from build123d import *

# Parameters (mm, degrees)
BOSS_EXTRUDE1_DEPTH = 6


with BuildPart() as part:
    # Sketch1 → Boss-Extrude1 (new body)
    with BuildSketch(Plane.XY):
        with BuildLine():
            Line((23.424737155, -30.334071959), (17.293543757, -15.098809177))
            ThreePointArc((17.293543757, -15.098809177), (16.817822135, -14.397549548), (16.094423456, -13.956221462))
            Line((16.094423456, -13.956221462), (15.963008089, -14.561962892))
            ThreePointArc((15.963008089, -14.561962892), (16.131735441, -17.04624853), (14.064088238, -15.658812373))
            Line((14.064088238, -15.658812373), (13.483620184, -15.421447711))
            ThreePointArc((13.483620184, -15.421447711), (13.445284936, -16.014246024), (13.582760132, -16.592156052))
            Line((13.582760132, -16.592156052), (19.41043004, -31.073200227))
            Line((19.41043004, -31.073200227), (19.719217872, -30.321121581))
            ThreePointArc((19.719217872, -30.321121581), (21.576335078, -29.08075761), (23.424737155, -30.334071959))
        make_face()
        with BuildLine():
            ThreePointArc((23.419472814, -31.840369211), (23.569333129, -31.087735131), (23.424737155, -30.334071959))
            ThreePointArc((23.424737155, -30.334071959), (21.576335078, -29.08075761), (19.719217872, -30.321121581))
            Line((19.719217872, -30.321121581), (19.41043004, -31.073200227))
            Line((19.41043004, -31.073200227), (19.71395353, -31.827418834))
            ThreePointArc((19.71395353, -31.827418834), (21.562355608, -33.080733182), (23.419472814, -31.840369211))
        make_face()
        with BuildLine():
            Line((18.045273154, -44.929682928), (23.419472814, -31.840369211))
            ThreePointArc((23.419472814, -31.840369211), (21.562355608, -33.080733182), (19.71395353, -31.827418834))
            Line((19.71395353, -31.827418834), (19.41043004, -31.073200227))
            Line((19.41043004, -31.073200227), (14.345018212, -43.410435298))
            Line((14.345018212, -43.410435298), (8.266248414, -50.481735298))
            ThreePointArc((8.266248414, -50.481735298), (14.114121661, -49.393703769), (18.045273154, -44.929682928))
        make_face()
    extrude(amount=BOSS_EXTRUDE1_DEPTH)


solid = part.part
Check sheet for the modelled part. Datum: model origin and axes. Units: mm. A direction names the side the tool comes from. Round coordinates to 2 decimals unless told otherwise and drop trailing zeros. Loops run counter-clockwise (first coordinate to the right, second up) from the corner with the lowest first, then second, coordinate; pieces in that order, holes last. Notation, with made-up numbers: M 65,-40 L 103,-40 A21 ccw 103,-1 Z; hole C 21.25,76 d5. An arc over 180 degrees is marked long. One line per question, with ' | ' between items. Start each with the question number.
Item 1: Gauge pin test, flat ends, axial feed: pin 1 Ø1.7 at (x, y) = (15.44, -15.85) entering from -Z; pin 2 Ø3 at (x, z) = (11.5, 4) entering from +Y; pin 3 Ø2 at (y, z) = (-44.5, 2.5) entering from -X; pin 4 Ø3 at (y, z) = (-46.5, 1.5) entering from +X. Record the tip position at first contact, or that the pin passes through.
Item 2: Section check D-D (y = -47). Record the boundary of the cut face in (x, z), and give its area (3 significant figures).
Item 3: Section check A-A (x = 19). Record the boundary of the cut face in (y, z).
Item 4: Section check C-C (x = 15). Record the boundary of the cut face in (y, z).
Item 5: Section check B-B (z = 2.4). Record the boundary of the cut face in (x, y).
Item 6: Set-up check for faces 5 (the face through (16.456, -23.731, 2.958)), 6 (the face through (16.83, -14.41, 2.96)): record each of +Z, -Z, +X, -X, +Y, -Y from which the full face is reachable in a straight line by a thin tool's end or side.
Item 7: Scan lines: probe 1 along Y at (x, z) = (16.25, 1.7); probe 2 along Y at (x, z) = (15.25, 3.4); probe 3 along Y at (x, z) = (17, 4.4). Record each from-to range of solid material in increasing order.
Item 8: Release check for a two-part mould opening along Y. For faces 1 (the face through (20.695, -38.477, 2.958)), 2 (the face through (20.4, -22.82, 2.96)), 3 (the face through (16.169, -17.024, 2.958)), 4 (the face through (23.57, -31.1, 2.96)) record: released by +Y, released by -Y, zero draft, split by the parting line, or undercut.
Worked out:
1) pin 1: through | pin 2: y = -44.98 | pin 3: x = 12.55 | pin 4: x = 18.02
2) outline: M 11.26,0 L 16.86,0 L 16.86,6 L 11.26,6 Z | area: 33.6 mm^2
3) outline: M -42.6,0 L -32.07,0 L -32.07,6 L -42.6,6 Z; M -30.05,0 L -19.34,0 L -19.34,6 L -30.05,6 Z
4) outline: M -48.82,0 L -41.82,0 L -41.82,6 L -48.82,6 Z; M -20.11,0 L -17.16,0 L -17.16,6 L -20.11,6 Z
5) outline: M 8.27,-50.48 A9.11 ccw 18.05,-44.93 L 23.42,-31.84 A2 ccw 23.42,-30.33 L 17.29,-15.1 A2 ccw 16.09,-13.96 L 15.96,-14.56 A1.39 cw long 14.06,-15.66 L 13.48,-15.42 A2 ccw 13.58,-16.59 L 19.41,-31.07 L 14.35,-43.41 Z
6) face 5: +Z, -Z, -X | face 6: +Z, -Z, +X, +Y
7) probe 1: -47.72 to -38.77, -23.22 to -16.97, -14.72 to -14.02 | probe 2: -48.63 to -41.21, -20.74 to -17.22 | probe 3: -46.81 to -36.94, -25.08 to -14.6
8) face 1: released by -Y | face 2: released by +Y | face 3: undercut | face 4: split by the parting line
